from build123d import *

# Parameters (mm, degrees)
SKETCH1_R           = 6
BOSS_EXTRUDE1_DEPTH = 33
SKETCH2_W           = 2
SKETCH2_H           = 2
CUT_EXTRUDE1_DEPTH  = 33
SKETCH3_R           = 1.5
CUT_EXTRUDE2_DEPTH  = 23
SKETCH4_R           = 1
CUT_EXTRUDE3_DEPTH  = 7
SKETCH5_R           = 3.5
CUT_EXTRUDE4_DEPTH  = 2
SKETCH6_R           = 3.4
BOSS_EXTRUDE2_DEPTH = 2


with BuildPart() as part:
    # Sketch1 → Boss-Extrude1 (new body)
    with BuildSketch(Plane.XY):
        Circle(SKETCH1_R)
    extrude(amount=BOSS_EXTRUDE1_DEPTH)

    # Sketch2 → Cut-Extrude1 (cut)
    with BuildSketch(Plane.XY.offset(33)):
        with Locations((0, 6)):
            Rectangle(SKETCH2_W, SKETCH2_H)
    cut_extrude1 = extrude(amount=-CUT_EXTRUDE1_DEPTH, mode=Mode.SUBTRACT)

    # Mirror1: Cut-Extrude1 across plane
    add(cut_extrude1.mirror(Plane.ZX), mode=Mode.SUBTRACT)

    # Sketch3 → Cut-Extrude2 (cut)
    with BuildSketch(Plane.XY.offset(33)):
        Circle(SKETCH3_R)
    extrude(amount=-CUT_EXTRUDE2_DEPTH, mode=Mode.SUBTRACT)

    # Sketch4 → Cut-Extrude3 (cut)
    with BuildSketch(Plane(origin=(0, 5, 0), x_dir=(1, 0, 0), z_dir=(0, 1, 0))):
        with Locations(Location((0, -7, 0), (0, 0, 270))):
            Circle(SKETCH4_R)
    extrude(amount=-CUT_EXTRUDE3_DEPTH, mode=Mode.SUBTRACT)

    # Sketch5 → Cut-Extrude4 (cut)
    with BuildSketch(Plane(origin=(0, 0, 0), x_dir=(-1, 0, 0), z_dir=(0, 0, -1))):
        Circle(SKETCH5_R)
    extrude(amount=-CUT_EXTRUDE4_DEPTH, mode=Mode.SUBTRACT)

    # Sketch6 → Boss-Extrude2 (add)
    with BuildSketch(Plane(origin=(0, 0, 2), x_dir=(-1, 0, 0), z_dir=(0, 0, -1))):
        with Locations(Location((0, 0, 0), (0, 0, 180))):
            Circle(SKETCH6_R)
    extrude(amount=BOSS_EXTRUDE2_DEPTH)


solid = part.part
Geometry check sheet. Reference: the model listing, model coordinates, mm. A direction names the side the tool comes from. Round coordinates to 2 decimals unless told otherwise and drop trailing zeros. Write each loop counter-clockwise with the first axis right and the second up, starting at its lowest first coordinate (ties: lowest second). Pieces come first, ordered by that corner, then holes. Notation, with made-up numbers: (7.5, 57.5) - (12.5, 57.5) arc R8 ccw to (12.5, 64.5) - close; hole circle Ø2 at (-13.5, 37). An arc over 180 degrees is marked (long way). One line per item, written item: value.
1. Mould release check, pull along X, two halves, no side actions. Record for faces 4 (the face through (-6, 0, 16)), 5 (the face through (0, 0, 10)), 6 (the face through (1.2, -1.2, 33)): released by +X, released by -X, zero draft, split by the parting line, or undercut.
The answers:
face 4: released by -X
face 5: undercut
face 6: zero draft
2. Cross-section at A-A on z = 29. Record the boundary of the cut face in (x, y), and give its area (3 significant figures).
The answers:
outline: (-1, -5.92) - (-1, -5) - (1, -5) - (1, -5.92) arc R6 ccw to (1, 5.92) - (1, 5) - (-1, 5) - (-1, 5.92) arc R6 ccw to start; hole circle Ø3 at (0, 0)
area: 102 mm^2
3. Set-up check for faces 1 (the face through (-1, -5.5, 16.7)), 2 (the face through (-0.6, 1.5, 6.2)), 3 (the face through (-1.5, 0.07, 21.66)): record each of +Z, -Z, +X, -X, +Y, -Y from which the full face is reachable in a straight line by a thin tool's end or side.
The answers:
face 1: +Z, -Z, -Y
face 2: +Y
face 3: +Z
4. Scan lines: L1, parallel to Z at x = 0, y = -0.5; L2, parallel to Y at x = 0, z = 14; L3, parallel to Z at x = 0, y = 2. Record each from-to range of solid material in increasing order.
The answers:
L1: z = 0 to 6, 8 to 10
L2: y = -5 to -1.5, 1.5 to 5
L3: z = 0 to 6, 8 to 33
5. Cross-section at C-C on z = 5.5. Record the boundary of the cut face in (x, y).
The answers:
outline: (-1, -5.92) - (-1, -5) - (1, -5) - (1, -5.92) arc R6 ccw to (1, 5.92) - (1, 5) - (-1, 5) - (-1, 5.92) arc R6 ccw to start
6. Depth check by flat-ended pin: pin 1 Ø0.6 at (x, z) = (0, 7) entering from +Y; pin 2 Ø4 at (y, z) = (2.5, 25) entering from -X; pin 3 Ø0.9 at (x, y) = (-0.5, 0.5) entering from +Z. Enter the tip coordinate at first touch or a pass-through.
The answers:
pin 1: stops at y = -2
pin 2: stops at x = -5.98
pin 3: stops at z = 10
7. Cross-section at D-D on x = 0. Record the boundary of the cut face in (y, z).
The answers:
outline: (-5, 0) - (-3.5, 0) - (-3.5, 2) - (-3.4, 2) - (-3.4, 0) - (3.4, 0) - (3.4, 2) - (3.5, 2) - (3.5, 0) - (5, 0) - (5, 6) - (-2, 6) - (-2, 8) - (5, 8) - (5, 33) - (1.5, 33) - (1.5, 10) - (-1.5, 10) - (-1.5, 33) - (-5, 33) - close
8. Cross-section at B-B on y = 0. Record the boundary of the cut face in (x, z), and give its area (3 significant figures).
The answers:
outline: (-6, 0) - (-3.5, 0) - (-3.5, 2) - (-3.4, 2) - (-3.4, 0) - (3.4, 0) - (3.4, 2) - (3.5, 2) - (3.5, 0) - (6, 0) - (6, 33) - (1.5, 33) - (1.5, 10) - (-1.5, 10) - (-1.5, 33) - (-6, 33) - close; hole circle Ø2 at (0, 7)
area: 323 mm^2
